```python
from build123d import *

# Parameters (mm, degrees)
SKETCH_1_W              = 40
SKETCH_1_H              = 50
EXTRUDE_1_DEPTH         = 10
SKETCH_2_R              = 12
CUT_EXTRUDE_1_DEPTH     = 6
SKETCH_3_R              = 8
CUT_EXTRUDE_2_DEPTH     = 33.57299495
HOLE_WIZARD_M4_1_D      = 3.3
HOLE_WIZARD_M4_1_DEPTH  = 10
HOLE_WIZARD_M4_1_TIP    = 0.991420021
FILLET_1_R              = 10
HOLE_WIZARD_M4_3_REACH  = 56.772
HOLE_WIZARD_M4_3_BORE_R = 1.65


with BuildPart() as part:
    # 草图1 → 凸台-拉伸1 (new body)
    with BuildSketch(Plane.XY):
        Rectangle(SKETCH_1_W, SKETCH_1_H)
    extrude(amount=EXTRUDE_1_DEPTH)

    # 草图2 → 切除-拉伸1 (cut)
    with BuildSketch(Plane.XY.offset(10)):
        with Locations((0, -5)):
            Circle(SKETCH_2_R)
    extrude(amount=-CUT_EXTRUDE_1_DEPTH, mode=Mode.SUBTRACT)

    # 草图3 → 切除-拉伸2 (cut, through all)
    with BuildSketch(Plane.XY.offset(4)):
        with Locations((0, -5)):
            Circle(SKETCH_3_R)
    extrude(amount=-CUT_EXTRUDE_2_DEPTH, mode=Mode.SUBTRACT)

    # M4 螺纹孔1
    with Locations(Plane(origin=(0, 25, 0), x_dir=(1, 0, 0), z_dir=(0, 1, 0))):
        with Locations((-15, -5), (15, -5)):
            Hole(HOLE_WIZARD_M4_1_D / 2, depth=HOLE_WIZARD_M4_1_DEPTH)
            with Locations((0, 0, -(HOLE_WIZARD_M4_1_DEPTH + HOLE_WIZARD_M4_1_TIP / 2))):  # 118° drill point
                Cone(0, HOLE_WIZARD_M4_1_D / 2, HOLE_WIZARD_M4_1_TIP, mode=Mode.SUBTRACT)

    # 圆角1
    fillet_1_edges = [part.edges().sort_by_distance(p)[0] for p in [
        (20, -25, 5),
        (-20, -25, 5),
    ]]
    fillet(fillet_1_edges, radius=FILLET_1_R)

    # M4 螺纹孔3 bore → M4 螺纹孔3 (cut, up to next)
    with BuildSketch(Plane(origin=(0, 25, 0), x_dir=(1, 0, 0), z_dir=(0, 1, 0)), mode=Mode.PRIVATE) as hole_wizard_m4_3_sk1:
        with Locations((0, -7)):
            Circle(HOLE_WIZARD_M4_3_BORE_R)
    hole_wizard_m4_3_tool1 = extrude(hole_wizard_m4_3_sk1.sketch, amount=-HOLE_WIZARD_M4_3_REACH, mode=Mode.PRIVATE) & part.part
    add(hole_wizard_m4_3_tool1.solids().sort_by_distance((0, 25, 7))[0], mode=Mode.SUBTRACT)


solid = part.part
```
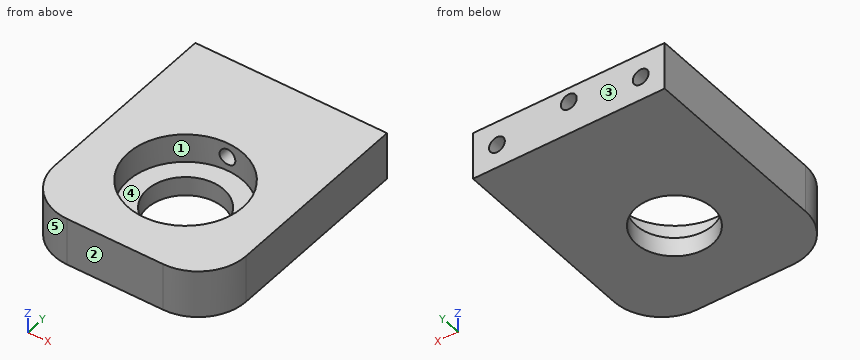
Could you check a few things on this model? Use its own coordinates, in mm. Face numbers are marked on the shaded views. A direction names the side the tool comes from. Coordinates: 2 decimals unless noted, no trailing zeros. Write each loop counter-clockwise with the first axis right and the second up, starting at its lowest first coordinate (ties: lowest second). Pieces come first, ordered by that corner, then holes. Notation, with made-up numbers: (24, -25.5) - (62, -25.5) arc R29 ccw to (62, -4.5) - close; hole circle Ø6 at (89.25, -20). An arc over 180 degrees is marked (long way). Use a Markdown table: item, result.
Q1. Imagine slicing it at B-B (y = -5). List the corners of the cut face in (x, z) for me.
Geometry check:
| item | result |
|---|---|
| outline | (-20, 0) - (-8, 0) - (-8, 4) - (-12, 4) - (-12, 10) - (-20, 10) - close; (8, 0) - (20, 0) - (20, 10) - (12, 10) - (12, 4) - (8, 4) - close |
Q2. Imagine slicing it at D-D (y = -18). List the corners of the cut face in (x, z) for me.
Geometry check:
| item | result |
|---|---|
| outline | (-19.54, 0) - (19.54, 0) - (19.54, 10) - (-19.54, 10) - close |
Q3. I'm going to push flat-ended pins straight in: pin 1 Ø13 at (x, y) = (0, -5) entering from -Z; pin 2 Ø3 at (x, z) = (-15, 5) entering from -Y; pin 3 Ø2.5 at (x, z) = (15, 5) entering from -Y. Where does each tip first touch, or does it pass through?
Geometry check:
| item | result |
|---|---|
| pin 1 | passes through |
| pin 2 | stops at y = -24.37 |
| pin 3 | stops at y = -24.27 |
Q4. Which directions (+Z, -Z, +X, -X, +Y, -Y) give clear straight access to the entire face, cutting with the end or side of a thin tool? Please do the marked faces 1 and 2.
Geometry check:
| item | result |
|---|---|
| face 1 | +Z |
| face 2 | +Z, -Z, +X, -X, -Y |
Q5. Please list where these lines run through material, in increasing order: L1, parallel to X at y = 18.5, z = 5; L2, parallel to Y at x = 0, z = 2.7; L3, parallel to Z at x = 15, y = 20.
Geometry check:
| item | result |
|---|---|
| L1 | x = -20 to -16.65, -13.35 to 13.35, 16.65 to 20 |
| L2 | y = -25 to -13, 3 to 25 |
| L3 | z = 0 to 3.35, 6.65 to 10 |
Q6. Thinking about a two-plate mould opening in Y: for the marked faces 3, 4 and 5, which applies, +Y half, -Y half, draft (parallel to the pull), parting line (faces both ways), or undercut?
Geometry check:
| item | result |
|---|---|
| face 3 | +Y half |
| face 4 | undercut |
| face 5 | -Y half |
Q7. Imagine slicing it at A-A (x = 0). List the corners of the cut face in (y, z) for me, and give its area (3 significant figures).
Geometry check:
| item | result |
|---|---|
| outline | (-25, 0) - (-13, 0) - (-13, 4) - (-17, 4) - (-17, 10) - (-25, 10) - close; (3, 0) - (25, 0) - (25, 5.35) - (7, 5.35) - (7, 4) - (3, 4) - close; (7, 8.65) - (25, 8.65) - (25, 10) - (7, 10) - close |
| area | 233 mm2 |
Q8. Imagine slicing it at C-C (x = -5.5). List the corners of the cut face in (y, z) for me.
Geometry check:
| item | result |
|---|---|
| outline | (-25, 0) - (-10.81, 0) - (-10.81, 4) - (-15.67, 4) - (-15.67, 10) - (-25, 10) - close; (0.81, 0) - (25, 0) - (25, 10) - (5.67, 10) - (5.67, 4) - (0.81, 4) - close |
